Job drawing, mm, ordinate dimensions from the low corner. One solid piece. A direction names the side the tool comes from. Coordinates: 2 decimals unless noted, no trailing zeros. Order: outer loops, then holes, each group sorted by start corner. A loop starts at its lowest first (then second) coordinate and runs counter-clockwise, first axis right, second up. Notation, with made-up numbers: M -21,32 L -5,32 A11 cw -5,43 Z; hole C 28.25,45.25 d10. An arc over 180 degrees is marked long. Write item = value, one per line.
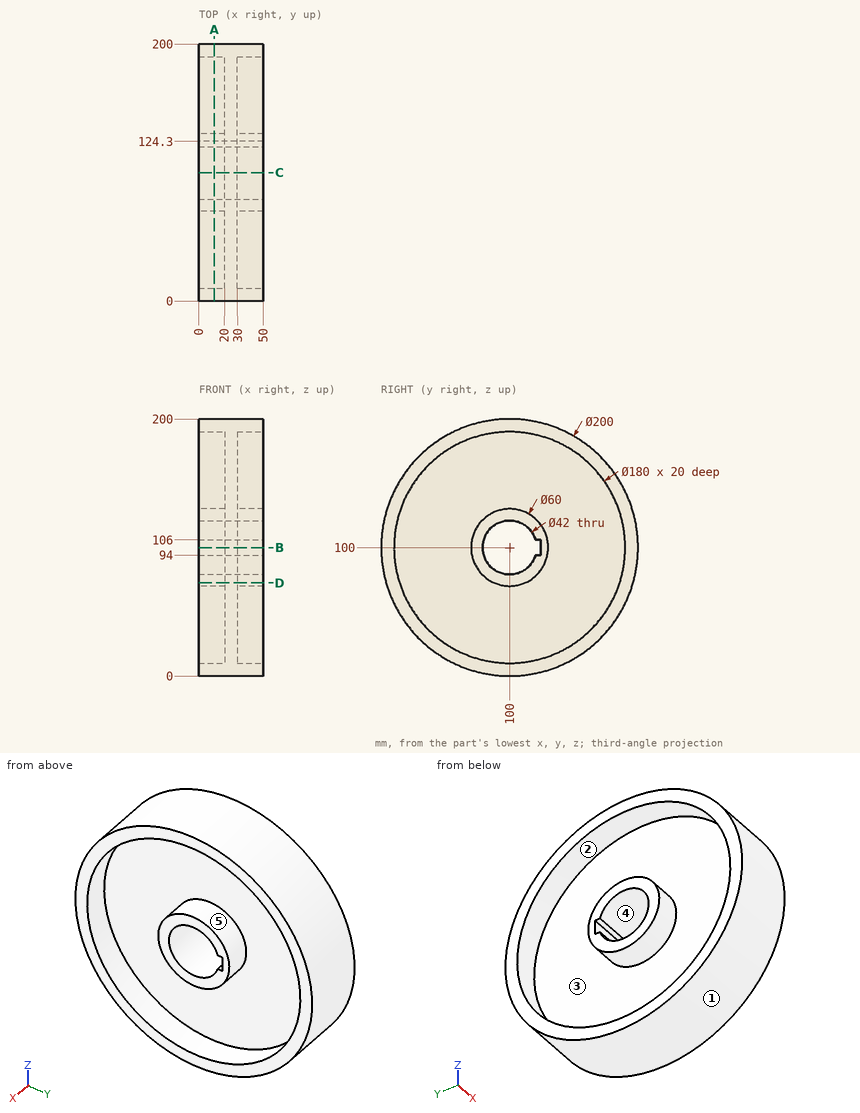
(1) Slice it at D-D, the plane z = 72.5. Write the cut outline in (x, y).
Evaluation:
outline = M 0,3.86 L 50,3.86 L 50,14.3 L 30,14.3 L 30,88.01 L 50,88.01 L 50,111.99 L 30,111.99 L 30,185.7 L 50,185.7 L 50,196.14 L 0,196.14 L 0,185.7 L 20,185.7 L 20,111.99 L 0,111.99 L 0,88.01 L 20,88.01 L 20,14.3 L 0,14.3 Z
(2) Slice it at B-B, the plane z = 100. Write the cut outline in (x, y).
Evaluation:
outline = M 0,0 L 50,0 L 50,10 L 30,10 L 30,70 L 50,70 L 50,79 L 0,79 L 0,70 L 20,70 L 20,10 L 0,10 Z; M 0,124.3 L 50,124.3 L 50,130 L 30,130 L 30,190 L 50,190 L 50,200 L 0,200 L 0,190 L 20,190 L 20,130 L 0,130 Z
(3) Wall check: line 1 (Y direction, x = 35, z = 100); line 2 (Y direction, x = 15, z = 124.5); line 3 (Y direction, x = 11, z = 81.5). Give the ranges that are in metal, low to high. Write a range as from..to.
Evaluation:
line_1 = 0..10, 70..79, 124.3..130, 190..200
line_2 = 3.05..13.4, 82.69..117.31, 186.6..196.95
line_3 = 1.73..11.92, 76.38..90.06, 109.94..123.62, 188.08..198.27
(4) Tool access for the marked faces 3, 4 and 5: list every direction of +Z, -Z, +X, -X, +Y, -Y with a clear straight run to the whole face (end or side of a thin tool).
Evaluation:
face_3 = -X
face_4 = +X, -X
face_5 = +X
(5) Slice it at A-A, the plane x = 12. Write the cut outline in (y, z), then the cut area to 3 significant figures.
Evaluation:
outline = C 100,100 d200; C 100,100 d60; hole C 100,100 d180; hole M 120.12,94 L 124.3,94 L 124.3,106 L 120.12,106 A21 ccw long Z
area = 7,370 mm²
(6) Slice it at C-C, the plane y = 100. Write the cut outline in (x, z).
Evaluation:
outline = M 0,0 L 50,0 L 50,10 L 30,10 L 30,70 L 50,70 L 50,79 L 0,79 L 0,70 L 20,70 L 20,10 L 0,10 Z; M 0,121 L 50,121 L 50,130 L 30,130 L 30,190 L 50,190 L 50,200 L 0,200 L 0,190 L 20,190 L 20,130 L 0,130 Z
(7) Pull direction Z, two halves, no side cores. Call the marked faces 1 and 2: +Z half, -Z half, draft (parallel to the pull), parting line (faces both ways), or undercut.
Evaluation:
face_1 = parting line
face_2 = undercut
(8) Pin check, flat tips, straight feed: pin 1 Ø12 at (x, z) = (44, 138) entering from +Y; pin 2 Ø6 at (x, z) = (37, 120) entering from -Y; pin 3 Ø8 at (x, z) = (43, 135.5) entering from -Y. Stop position of each tip, or through.
Evaluation:
pin_1 = 194.74
pin_2 = 1.46
pin_3 = 5.09
